The model under review builds one solid part; all positions refer to its coordinate system, in mm. Face numbers are marked on the shaded views. Round coordinates to 2 decimals unless told otherwise and drop trailing zeros. Write each loop counter-clockwise with the first axis right and the second up, starting at its lowest first coordinate (ties: lowest second). Pieces come first, ordered by that corner, then holes. Notation, with made-up numbers: M -20.5,-35.5 L -6.5,-35.5 A16 ccw -6.5,-23.5 Z; hole C 37.25,71 d7. An arc over 180 degrees is marked long. Write item = value, one per line. Start each with the question number.
Item 1: For pin 1 Ø8 at (x, z) = (-25, 0) entering from -Y, flat-tipped, find the tip position at first contact; note if it passes through.
Item 2: Take a section at B-B, the plane z = 0. Give the boundary of the cut face in (x, y), plus the area to 3 significant figures.
Item 3: Take a section at C-C, the plane y = 0.35. Give the boundary of the cut face in (x, z), plus the area to 3 significant figures.
Item 4: Take a section at A-A, the plane x = 1.5. Give the boundary of the cut face in (y, z), plus the area to 3 significant figures.
Item 5: To check wall thickness, follow line 1 along Z through (x, y) = (0, -1.05); line 2 along X through (y, z) = (1, 1.25); line 3 along X through (y, z) = (-0.85, 0.75). State the ranges of each line that lie inside material, in increasing order.
Item 6: The part is to be moulded in two halves that separate along X. For the marked faces 1 and 2, say which applies: +X half, -X half, draft (parallel to the pull), parting line (faces both ways), or undercut.
from build123d import *

# Parameters (mm, degrees)
SKETCH_2_W         = 65
SKETCH_2_H         = 14
EXTRUDE_1_DEPTH    = 2
HOLE_WIZARD_M6_1_D = 5


with BuildPart() as part:
    # 草图2 → 凸台-拉伸1 (new, symmetric)
    with BuildSketch(Plane(origin=(0, 0, 0), x_dir=(1, 0, 0), z_dir=(0, 1, 0))):
        Rectangle(SKETCH_2_W, SKETCH_2_H)
    extrude(amount=EXTRUDE_1_DEPTH, both=True)

    # M6 螺纹孔1 (through all)
    with Locations(Plane(origin=(0, 2, 0), x_dir=(1, 0, 0), z_dir=(0, 1, 0))):
        with Locations((-25, 0), (0, 0), (25, 0)):
            Hole(HOLE_WIZARD_M6_1_D / 2)


solid = part.part
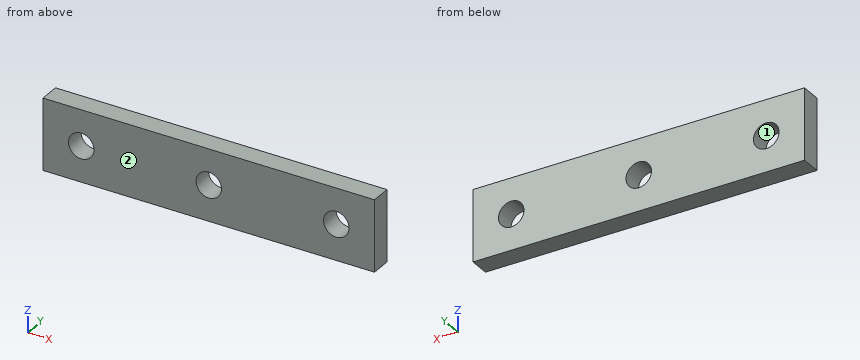
Response values:
q1.pin_1 = -2
q2.outline = M -32.5,-2 L -27.5,-2 L -27.5,2 L -32.5,2 Z; M -22.5,-2 L -2.5,-2 L -2.5,2 L -22.5,2 Z; M 2.5,-2 L 22.5,-2 L 22.5,2 L 2.5,2 Z; M 27.5,-2 L 32.5,-2 L 32.5,2 L 27.5,2 Z
q2.area = 200 mm2
q3.outline = M -32.5,-7 L 32.5,-7 L 32.5,7 L -32.5,7 Z; hole C -25,0 d5; hole C 0,0 d5; hole C 25,0 d5
q3.area = 851 mm2
q4.outline = M -2,-7 L 2,-7 L 2,-2 L -2,-2 Z; M -2,2 L 2,2 L 2,7 L -2,7 Z
q4.area = 40.0 mm2
q5.line_1 = -7 to -2.5, 2.5 to 7
q5.line_2 = -32.5 to -27.17, -22.83 to -2.17, 2.17 to 22.83, 27.17 to 32.5
q5.line_3 = -32.5 to -27.38, -22.62 to -2.38, 2.38 to 22.62, 27.38 to 32.5
q6.face_1 = undercut
q6.face_2 = draft
